Here's how the part is built. I have some questions about the finished solid (model axes, mm). A direction names the side the tool comes from. Coordinates: 2 decimals unless noted, no trailing zeros. Order: outer loops, then holes, each group sorted by start corner. A loop starts at its lowest first (then second) coordinate and runs counter-clockwise, first axis right, second up. Notation, with made-up numbers: (-6, 45.5) - (22, 45.5) arc R14 cw to (22, 61.5) - close; hole circle Ø4 at (76, 25.25). An arc over 180 degrees is marked (long way). Answer in a Markdown table with one row per item. Add a question column.
Item 1: If I drill on line 1 along Y through (x, z) = (10, 3); line 2 along X through (y, z) = (-20, 55); line 3 along Y through (x, z) = (28, 18), over which ranges is the centre line in solid material (lowest first)? Write a range as from..to.
Item 2: I want a section at A-A (y = -19). Please give me the cut outline in (x, z).
Item 3: Thinking about a two-plate mould opening in X: for faces 3 (the cylindrical face through (56, -38, 5)), 4 (the cylindrical face through (2.85, -46.99, 4.93)), 5 (the flat face through (16, -25, 55)), 6 (the cylindrical face through (14.619, -36.915, 5.07)), which applies, +X half, -X half, draft (parallel to the pull), parting line (faces both ways), or undercut?
Item 4: On a 3-axis mill with a long thin cutter (end or side, diameter ignored), from which of +Z, -Z, +X, -X, +Y, -Y can I reach the whole of each face in a straight line? I mean faces 1 (the cylindrical face through (5, -13, 65)), 2 (the flat face through (0, -20, 5)). Say none if no direction works.
Item 5: Will these pins go through, and if not, where does the flat tip stop? pin 1 Ø10 at (x, y) = (33, -28.5) entering from +Z; pin 2 Ø10 at (x, z) = (23.5, 50) entering from -Y; pin 3 Ø8 at (y, z) = (-24, 4.5) entering from -X.
Item 6: I want a section at B-B (y = -35). Please give me the cut outline in (x, z), plus the area to 3 significant figures.
Item 7: I want a section at C-C (z = 55). Please give me the cut outline in (x, y), plus the area to 3 significant figures.
Item 8: I want a section at D-D (z = 39.5). Please give me the cut outline in (x, y), plus the area to 3 significant figures.
```python
from build123d import *

# Parameters (mm, degrees)
BASE_PLATE_DEPTH         = 10
SIDE_PLATE_DEPTH         = 10
HUB_BOSS_SKETCH_R        = 17.5
HUB_BOSS_35_DEPTH        = 15
HUB_BORE_SKETCH_R        = 10
HUB_BORE_20_DEPTH        = 25
SIDE_PLATE_HOLE_SKETCH_R = 5
SIDE_PLATE_HOLE_DEPTH    = 10


with BuildPart() as part:
    # Base Plate Sketch → Base Plate (new body)
    with BuildSketch(Plane.XY):
        with BuildLine():
            Line((0, 0), (0, -40))
            ThreePointArc((0, -40), (2.928932188, -47.071067812), (10, -50))
            Line((10, -50), (60, -50))
            ThreePointArc((60, -50), (67.071067812, -47.071067812), (70, -40))
            Line((70, -40), (70, 0))
            Line((70, 0), (0, 0))
        make_face()
    extrude(amount=BASE_PLATE_DEPTH)

    # Side Plate Sketch → Side Plate (add)
    with BuildSketch(Plane(origin=(0, 0, 0), x_dir=(1, 0, 0), z_dir=(0, 1, 0))):
        with BuildLine():
            Line((18.565158101, -66.056061039), (70, -10))
            Line((70, -10), (0, -10))
            Line((0, -10), (-11.072048142, -48.076181073))
            ThreePointArc((-11.072048142, -48.076181073), (8.534767144, -37.860705346), (22.5, -55))
            ThreePointArc((22.5, -55), (21.486968593, -60.867696875), (18.565158101, -66.056061039))
        make_face()
        with BuildLine():
            Line((17.179494078, -67.566221548), (18.565158101, -66.056061039))
            ThreePointArc((18.565158101, -66.056061039), (21.486968593, -60.867696875), (22.5, -55))
            ThreePointArc((22.5, -55), (8.534767144, -37.860705346), (-11.072048142, -48.076181073))
            Line((-11.072048142, -48.076181073), (-12.278719231, -52.225858378))
            ThreePointArc((-12.278719231, -52.225858378), (-3.08283427, -70.52152667), (17.179494078, -67.566221548))
        make_face()
    extrude(amount=-SIDE_PLATE_DEPTH)

    # Hub Boss Sketch → Hub Boss Ø35 (add)
    with BuildSketch(Plane.XZ.offset(10)):
        with Locations(Location((5, 55, 0), (0, 0, 45.895348857))):
            Circle(HUB_BOSS_SKETCH_R)
    extrude(amount=HUB_BOSS_35_DEPTH)

    # Hub Bore Sketch → Hub Bore Ø20 (cut)
    with BuildSketch(Plane.XZ.offset(25)):
        with Locations(Location((5, 55, 0), (0, 0, 270))):
            Circle(HUB_BORE_SKETCH_R)
    extrude(amount=-HUB_BORE_20_DEPTH, mode=Mode.SUBTRACT)

    # Side Plate Hole Sketch → Side Plate Hole (cut)
    with BuildSketch(Plane.XY.offset(10)):
        with Locations((10, -35)):
            Circle(SIDE_PLATE_HOLE_SKETCH_R)
        with Locations((60, -35)):
            Circle(SIDE_PLATE_HOLE_SKETCH_R)
    extrude(amount=-SIDE_PLATE_HOLE_DEPTH, mode=Mode.SUBTRACT)


solid = part.part
```
Values follow:
| question | item | result |
|---|---|---|
| 1 | line 1 | y = -50..-40, -30..0 |
| 1 | line 2 | x = -12.5..-5, 15..22.5 |
| 1 | line 3 | y = -10..0 |
| 2 | outline | circle Ø35 at (5, 55); (0, 0) - (70, 0) - (70, 10) - (0, 10) - close; hole circle Ø20 at (5, 55) |
| 3 | face 3 | undercut |
| 3 | face 4 | -X half |
| 3 | face 5 | draft |
| 3 | face 6 | undercut |
| 4 | face 1 | +Y, -Y |
| 4 | face 2 | -Z, -X, +Y, -Y |
| 5 | pin 1 | stops at z = 10 |
| 5 | pin 2 | stops at y = -25 |
| 5 | pin 3 | stops at x = 0 |
| 6 | outline | (0, 0) - (5, 0) - (5, 10) - (0, 10) - close; (15, 0) - (55, 0) - (55, 10) - (15, 10) - close; (65, 0) - (70, 0) - (70, 10) - (65, 10) - close |
| 6 | area | 500 mm^2 |
| 7 | outline | (-12.5, -25) - (-5, -25) - (-5, 0) - (-12.5, 0) - close; (15, -25) - (22.5, -25) - (22.5, -10) - (28.71, -10) - (28.71, 0) - (15, 0) - close |
| 7 | area | 437 mm^2 |
| 8 | outline | (-8.58, -10) - (-3.12, -10) - (-3.12, -25) - (13.12, -25) - (13.12, -10) - (42.93, -10) - (42.93, 0) - (-8.58, 0) - close |
| 8 | area | 759 mm^2 |
